Build history of the part. All positions in model axes, mm. Face numbers are marked on the shaded views. A direction names the side the tool comes from. Give positions to 0.01 mm unless a question says otherwise; leave off trailing zeros. Loops run counter-clockwise (first coordinate to the right, second up) from the corner with the lowest first, then second, coordinate; pieces in that order, holes last. Notation, with made-up numbers: (41, 48) -> (46, 48) arc R18 cw to (46, 63) -> close; hole circle Ø1 at (8.5, 78.5). An arc over 180 degrees is marked (long way). Answer as a JSON object with one key per item and string values. Group by question number.
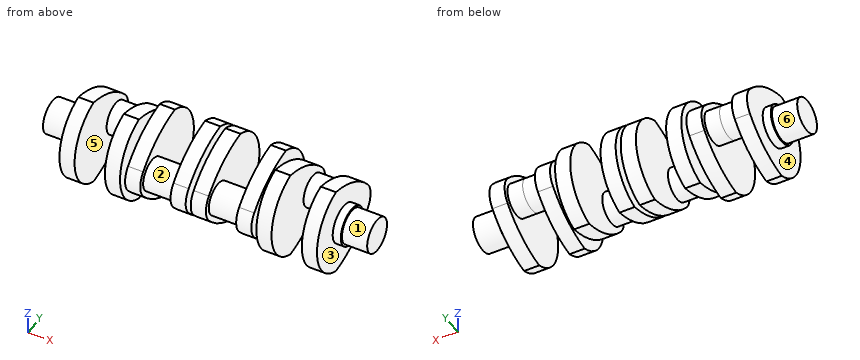
from build123d import *

# Parameters (mm, degrees)
END_JOURNAL_PROFILE_R         = 17
END_JOURNAL_34_DEPTH          = 25
SKETCH1_3_R                   = 19
JOURNAL_COLLAR_38_DEPTH       = 8
CRANK_WEB_1_DEPTH             = 15
CRANK_PIN_1_PROFILE_R         = 16
CRANK_PIN_1_32_DEPTH          = 15
MAIN_START                    = 5
MAIN_JOURNAL_SPACER_PROFILE_R = 17
MAIN_JOURNAL_SPACER_34_DEPTH  = 5
CRANK_WEB_3_DEPTH             = 15
CRANK_PIN_2_PROFILE_R         = 16
CRANK_PIN_2_32_DEPTH          = 30
CRANK_WEB_4_DEPTH             = 15
CENTRE_START                  = 2.5
CENTRE_JOURNAL_PROFILE_R      = 17
CENTRE_JOURNAL_HALF_34_DEPTH  = 2.5


with BuildPart() as part:
    # End Journal Profile → End Journal _34 (new body)
    with BuildSketch(Plane(origin=(0, 0, 0), x_dir=(0, 0, -1), z_dir=(1, 0, 0))):
        Circle(END_JOURNAL_PROFILE_R)
    extrude(amount=-END_JOURNAL_34_DEPTH)

    # Sketch1_3 → Journal Collar _38 (add)
    with BuildSketch(Plane(origin=(0, 0, 0), x_dir=(0, 0, -1), z_dir=(1, 0, 0))):
        Circle(SKETCH1_3_R)
    extrude(amount=JOURNAL_COLLAR_38_DEPTH)

    # Crank Web 1 Profile → Crank Web 1 (add)
    with BuildSketch(Plane(origin=(8, 0, 0), x_dir=(0, 0, -1), z_dir=(1, 0, 0))):
        with BuildLine():
            ThreePointArc((13.668094758, 40.943123461), (0, 46), (-13.668094758, 40.943123461))
            ThreePointArc((-13.668094758, 40.943123461), (-33.683444249, 16.469257624), (-44, -13.416407865))
            ThreePointArc((-44, -13.416407865), (0, -46), (44, -13.416407865))
            ThreePointArc((44, -13.416407865), (33.683444249, 16.469257624), (13.668094758, 40.943123461))
        make_face()
    crank_web_1 = extrude(amount=CRANK_WEB_1_DEPTH)

    # Crank Pin 1 Profile → Crank Pin 1 _32 (add)
    with BuildSketch(Plane(origin=(23, 0, 0), x_dir=(0, 0, -1), z_dir=(1, 0, 0))):
        with Locations(Location((0, 25, 0), (0, 0, 180))):
            Circle(CRANK_PIN_1_PROFILE_R)
    crank_pin_1_32 = extrude(amount=CRANK_PIN_1_32_DEPTH)

    # Crank Web 2 Mirror: Crank Web 1, Crank Pin 1 _32 across plane
    add(crank_web_1.mirror(Plane(origin=(38, 25, 0), x_dir=(0, 0, 1), z_dir=(1, 0, 0))))
    add(crank_pin_1_32.mirror(Plane(origin=(38, 25, 0), x_dir=(0, 0, 1), z_dir=(1, 0, 0))))

    # Main Journal Spacer Profile → Main Journal Spacer _34 (add)
    with BuildSketch(Plane(origin=(68, 0, 0), x_dir=(0, 0, -1), z_dir=(1, 0, 0)).offset(MAIN_START)):
        Circle(MAIN_JOURNAL_SPACER_PROFILE_R)
    extrude(amount=-MAIN_JOURNAL_SPACER_34_DEPTH)

    # Crank Web 3 Profile → Crank Web 3 (add)
    with BuildSketch(Plane(origin=(73, 0, 0), x_dir=(0, 0, -1), z_dir=(1, 0, 0))):
        with BuildLine():
            ThreePointArc((-13.668094758, -40.943123461), (0, -46), (13.668094758, -40.943123461))
            ThreePointArc((13.668094758, -40.943123461), (33.683444249, -16.469257624), (44, 13.416407865))
            ThreePointArc((44, 13.416407865), (0, 46), (-44, 13.416407865))
            ThreePointArc((-44, 13.416407865), (-33.683444249, -16.469257624), (-13.668094758, -40.943123461))
        make_face()
    extrude(amount=CRANK_WEB_3_DEPTH)

    # Crank Pin 2 Profile → Crank Pin 2 _32 (add)
    with BuildSketch(Plane(origin=(88, 0, 0), x_dir=(0, 0, -1), z_dir=(1, 0, 0))):
        with Locations((0, -25)):
            Circle(CRANK_PIN_2_PROFILE_R)
    extrude(amount=CRANK_PIN_2_32_DEPTH)

    # Crank Web 4 Profile → Crank Web 4 (add)
    with BuildSketch(Plane(origin=(118, 0, 0), x_dir=(0, 0, -1), z_dir=(1, 0, 0))):
        with BuildLine():
            ThreePointArc((-13.668094758, -40.943123461), (0, -46), (13.668094758, -40.943123461))
            ThreePointArc((13.668094758, -40.943123461), (33.683444249, -16.469257624), (44, 13.416407865))
            ThreePointArc((44, 13.416407865), (0, 46), (-44, 13.416407865))
            ThreePointArc((-44, 13.416407865), (-33.683444249, -16.469257624), (-13.668094758, -40.943123461))
        make_face()
    extrude(amount=CRANK_WEB_4_DEPTH)

    # Centre Journal Profile → Centre Journal Half _34 (add)
    with BuildSketch(Plane(origin=(133, 0, 0), x_dir=(0, 0, -1), z_dir=(1, 0, 0)).offset(CENTRE_START)):
        Circle(CENTRE_JOURNAL_PROFILE_R)
    extrude(amount=-CENTRE_JOURNAL_HALF_34_DEPTH)

    # Crankshaft Half Mirror: part across plane


with BuildPart() as part_1:
    add(part.part)
    add(part.part.mirror(Plane(origin=(135.5, 0, 0), x_dir=(0, 0, 1), z_dir=(1, 0, 0))))


solid = part_1.part
(1) 3-axis set-ups, long thin cutter, end or side, ignore diameter. For the marked faces 1 and 2: which of +Z, -Z, +X, -X, +Y, -Y reach the whole face in a straight line?
(2) Probe line 1 along X through (y, z) = (11, -2); line 2 along X through (y, z) = (15.5, -37.5); line 3 along X through (y, z) = (32.5, -10). List the from-to ranges inside material, lowest first. Write a range as [from, to].
(3) Pull direction X, two halves, no side cores. Call the marked faces 3, 4, 5 and 6: pulls with the +X half, pulls with the -X half, needs draft (parallel to the pull), parting line crosses it, or undercut.
(4) Saw through at B-B on x = 77.5. List the corners of the cut face in (y, z), plus the area to 3 significant figures.
(5) Pin check, flat tips, straight feed: pin 1 (1.5 mm diameter, centred on y = -21, z = 27, fed in from -X); pin 2 (6 mm diameter, centred on x = 11.5, y = 6, fed in from +Z); pin 3 (10 mm diameter, centred on x = 182.5, y = -8, fed in from -Z). Stop position of each tip, or through.
(6) Saw through at A-A on z = 36. Give the number of separate pieces and of enclosed holes in the cut face, plus the area to 3 significant figures.
Calculated:
{
 "1": {"face 1": "+X", "face 2": "none"},
 "2": {"line 1": "x = [-25, 88], [118, 153], [183, 296]", "line 2": "x = [73, 88], [118, 133], [138, 153], [183, 198]", "line 3": "x = [8, 68], [73, 88], [118, 133], [138, 153], [183, 198], [203, 263]"},
 "3": {"face 3": "pulls with the +X half", "face 4": "pulls with the -X half", "face 5": "undercut", "face 6": "needs draft"},
 "4": {"outline": "(-40.94, -13.67) arc R90 ccw to (13.42, -44) arc R46 ccw to (13.42, 44) arc R90 ccw to (-40.94, 13.67) arc R21 ccw to start", "area": "5,800 mm^2"},
 "5": {"pin 1": "stops at x = 8", "pin 2": "stops at z = 39.81", "pin 3": "stops at z = -39.8"},
 "6": {"separate pieces": "8", "enclosed holes": "0", "area": "4,880 mm^2"}
}
